The listing builds one solid part. Answer for the finished solid, in the listing's coordinates (mm). A direction names the side the tool comes from. Round coordinates to 2 decimals unless told otherwise and drop trailing zeros. Write each loop counter-clockwise with the first axis right and the second up, starting at its lowest first coordinate (ties: lowest second). Pieces come first, ordered by that corner, then holes. Notation, with made-up numbers: (5.25, 31) - (16.25, 31) arc R11 cw to (16.25, 45) - close; hole circle Ø3 at (-15.5, 65). An arc over 180 degrees is marked (long way). Return JSON: item names as keys, results as strings. Group by question number.
from build123d import *

# Parameters (mm, degrees)
SKETCH_1_R          = 45
SKETCH_1_R_2        = 13.25
EXTRUDE_1_DEPTH     = 2
CUT_EXTRUDE_1_REACH = 65.765


with BuildPart() as part:
    # 草图1 → 凸台-拉伸1 (new, symmetric)
    with BuildSketch(Plane(origin=(0, 0, 0), x_dir=(1, 0, 0), z_dir=(0, 1, 0))):
        with Locations(Location((0, 0, 0), (0, 0, 270))):
            Circle(SKETCH_1_R)
        with Locations(Location((0, 0, 0), (0, 0, 270))):
            Circle(SKETCH_1_R_2, mode=Mode.SUBTRACT)
    extrude(amount=EXTRUDE_1_DEPTH, both=True)

    # 草图2 → 切除-拉伸1 (cut, up to next)
    with BuildSketch(Plane.XZ.offset(2), mode=Mode.PRIVATE) as cut_extrude_1_sk1:
        with BuildLine():
            Line((-13.23838441, 0.5546875), (-13.23838441, 3.5546875))
            ThreePointArc((-13.23838441, 3.5546875), (0, 32.5), (13.23838441, 3.5546875))
            Line((13.23838441, 3.5546875), (13.23838441, 0.5546875))
            Line((13.23838441, 0.5546875), (-13.23838441, 0.5546875))
        make_face()
    cut_extrude_1_tool1 = extrude(cut_extrude_1_sk1.sketch, amount=-CUT_EXTRUDE_1_REACH, mode=Mode.PRIVATE) & part.part
    add(cut_extrude_1_tool1.solids().sort_by_distance((0, -2, 15.557308))[0], mode=Mode.SUBTRACT)


solid = part.part
(1) Find section A-A (y = 1.2). Write down the section's boundary in (x, z), plus the area to 3 significant figures.
(2) Find section C-C (z = -3). Write down the section's boundary in (x, y), plus the area to 3 significant figures.
(3) Find section B-B (x = -7.5). Write down the section's boundary in (y, z), plus the area to 3 significant figures.
(4) Find section D-D (x = 19.5). Write down the section's boundary in (y, z), plus the area to 3 significant figures.
(5) Determine the mould class of faces 3 (the cylindrical face through (-0.56, -0.03, 32.49)), 4 (the flat face through (-9, 2, -11)), 5 (the cylindrical face through (-17.235, 0.028, 41.569)) for opening direction Z: +Z half, -Z half, draft (parallel to the pull), parting line (faces both ways), or undercut.
(6) Flat-ended cylindrical pins translate along their axes: pin 1 (21 mm diameter, centred on x = 0, z = 15, fed in from +Y); pin 2 (1.5 mm diameter, centred on x = -32.5, y = 1.5, fed in from +Z); pin 3 (1.5 mm diameter, centred on y = 0.5, z = -24.5, fed in from -X). Find the tip coordinate at first contact, or state that the pin passes through.
(7) Consider line 1 (X direction, y = -0.4, z = -1); line 2 (X direction, y = -0.25, z = 15); line 3 (Z direction, x = -14, y = 1.3). Determine where each line is inside the solid, lowest interval first.
(8) For faces 1 (the cylindrical face through (0.299, -0.028, -13.247)), 2 (the flat face through (-9, -2, -11)), determine the directions among +Z, -Z, +X, -X, +Y, -Y from which every point of the face is accessible in a straight line to the end or side of a thin tool.
Check sheet entries:
{
 "1": {"outline": "circle Ø90 at (0, 0); hole (-13.24, 0.55) arc R13.25 ccw (long way) to (13.24, 0.55) - (13.24, 3.55) arc R17.5 ccw (long way) to (-13.24, 3.55) - close", "area": "5,140 mm^2"},
 "2": {"outline": "(-44.9, -2) - (-12.91, -2) - (-12.91, 2) - (-44.9, 2) - close; (12.91, -2) - (44.9, -2) - (44.9, 2) - (12.91, 2) - close", "area": "256 mm^2"},
 "3": {"outline": "(-2, -44.37) - (2, -44.37) - (2, -10.92) - (-2, -10.92) - close; (-2, 30.81) - (2, 30.81) - (2, 44.37) - (-2, 44.37) - close", "area": "188 mm^2"},
 "4": {"outline": "(-2, -40.56) - (2, -40.56) - (2, 40.56) - (-2, 40.56) - close", "area": "324 mm^2"},
 "5": {"face 3": "undercut", "face 4": "draft", "face 5": "parting line"},
 "6": {"pin 1": "passes through", "pin 2": "stops at z = 31.89", "pin 3": "stops at x = -38.22"},
 "7": {"line 1": "x = -44.99 to -13.21, 13.21 to 44.99", "line 2": "x = -42.43 to -17.5, 17.5 to 42.43", "line 3": "z = -42.77 to 4.5, 25.5 to 42.77"},
 "8": {"face 1": "+Y, -Y", "face 2": "+Z, -Z, +X, -X, -Y"}
}
